Read the model definition and answer for the solid it produces. Units are mm, in the model's axes. Coordinates: 2 decimals unless noted, no trailing zeros. Write each loop counter-clockwise with the first axis right and the second up, starting at its lowest first coordinate (ties: lowest second). Pieces come first, ordered by that corner, then holes.
(1) Find the intervals of material crossed by probe 1 along X at (y, z) = (3.5, 92); probe 2 along Z at (x, y) = (-72, 3.5); probe 3 along X at (y, z) = (3.75, 6.5), in increasing order.
(2) Section C-C on z = 6.5 is taken. Write down the section's boundary in (x, y).
(3) Section D-D on x = 0 is taken. Write down the section's boundary in (y, z).
(4) Section A-A on z = 92 is taken. Write down the section's boundary in (x, y).
(5) Section B-B on x = 72 is taken. Write down the section's boundary in (y, z), then the cut area to 3 significant figures.
(6) Given pin 1 (10 mm diameter, centred on x = 37.5, z = 63.5, fed in from -Y), flat-ended and moving along its own axis, determine where the tip first touches the part or whether it passes through.
from build123d import *

# Parameters (mm, degrees)
SKETCH_1_W               = 170
SKETCH_1_H               = 210
EXTRUDE_1_DEPTH          = 10
CUT_EXTRUDE_1_REACH      = 137.462
SKETCH_2_R               = 9.5
CUT_EXTRUDE_2_REACH      = 137.462
SKETCH_3_R               = 3.5
MIRROR_2_COPY_1_REACH    = 137.462
MIRROR_2_COPY_1_SKETCH_R = 3.5
CHAMFER_1_SIZE           = 2


with BuildPart() as part:
    # 草图1 → 凸台-拉伸1 (new body)
    with BuildSketch(Plane(origin=(0, 0, 0), x_dir=(1, 0, 0), z_dir=(0, 1, 0))):
        Rectangle(SKETCH_1_W, SKETCH_1_H)
    extrude(amount=EXTRUDE_1_DEPTH)

    # 草图2 → 切除-拉伸1 (cut, up to next)
    with BuildSketch(Plane(origin=(0, 10, 0), x_dir=(1, 0, 0), z_dir=(0, 1, 0)), mode=Mode.PRIVATE) as cut_extrude_1_sk1:
        with Locations(Location((0, -6.5, 0), (0, 0, 270))):
            Circle(SKETCH_2_R)
    cut_extrude_1_tool1 = extrude(cut_extrude_1_sk1.sketch, amount=-CUT_EXTRUDE_1_REACH, mode=Mode.PRIVATE) & part.part
    add(cut_extrude_1_tool1.solids().sort_by_distance((0, 10, 6.5))[0], mode=Mode.SUBTRACT)

    # 草图3 → 切除-拉伸2 (cut, up to next)
    with BuildSketch(Plane.XZ, mode=Mode.PRIVATE) as cut_extrude_2_sk1:
        with Locations(Location((72, 92, 0), (0, 0, 270))):
            Circle(SKETCH_3_R)
    cut_extrude_2_tool1 = extrude(cut_extrude_2_sk1.sketch, amount=-CUT_EXTRUDE_2_REACH, mode=Mode.PRIVATE) & part.part
    cut_extrude_2 = cut_extrude_2_tool1.solids().sort_by_distance((72, 0, 92))[0]
    add(cut_extrude_2, mode=Mode.SUBTRACT)

    # 镜向1: 切除-拉伸2 across plane
    add(cut_extrude_2.mirror(Plane(origin=(0, 0, 0), x_dir=(0, 0, 1), z_dir=(1, 0, 0))), mode=Mode.SUBTRACT)

    # 镜向2: 切除-拉伸2 across plane
    add(cut_extrude_2.mirror(Plane.XY), mode=Mode.SUBTRACT)

    # 镜向2 copy 1 sketch → 镜向2 copy 1 (cut, up to next)
    with BuildSketch(Plane(origin=(0, 0, 0), x_dir=(-1, 0, 0), z_dir=(0, -1, 0)), mode=Mode.PRIVATE) as mirror_2_copy_1_sk1:
        with Locations(Location((72, 92, 0), (0, 0, 270))):
            Circle(MIRROR_2_COPY_1_SKETCH_R)
    mirror_2_copy_1_tool1 = extrude(mirror_2_copy_1_sk1.sketch, amount=-MIRROR_2_COPY_1_REACH, mode=Mode.PRIVATE) & part.part
    add(mirror_2_copy_1_tool1.solids().sort_by_distance((-72, 0, -92))[0], mode=Mode.SUBTRACT)

    # 倒角1
    chamfer_1_edges = [part.edges().sort_by_distance(p)[0] for p in [
        (85, 5, 105),
        (-85, 5, 105),
        (-85, 5, -105),
        (85, 5, -105),
    ]]
    chamfer(chamfer_1_edges, length=CHAMFER_1_SIZE)


solid = part.part
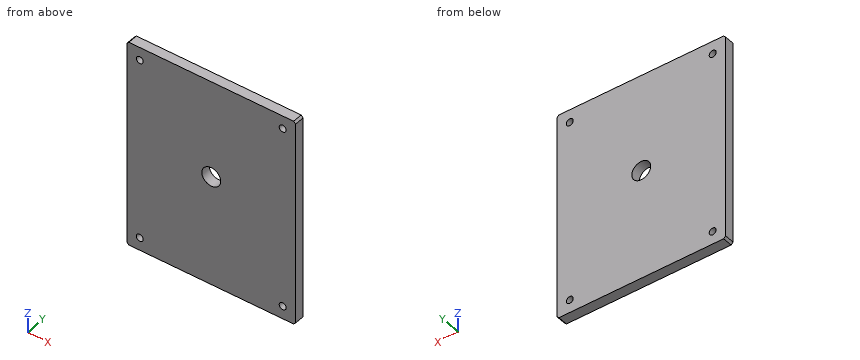
Response:
1. probe 1: x = -85 to -75.5, -68.5 to 68.5, 75.5 to 85
1. probe 2: z = -105 to -95.5, -88.5 to 88.5, 95.5 to 105
1. probe 3: x = -85 to -9.5, 9.5 to 85
2. outline: (-85, 0) - (-9.5, 0) - (-9.5, 10) - (-85, 10) - close; (9.5, 0) - (85, 0) - (85, 10) - (9.5, 10) - close
3. outline: (0, -105) - (10, -105) - (10, -3) - (0, -3) - close; (0, 16) - (10, 16) - (10, 105) - (0, 105) - close
4. outline: (-85, 0) - (-75.5, 0) - (-75.5, 10) - (-85, 10) - close; (-68.5, 0) - (68.5, 0) - (68.5, 10) - (-68.5, 10) - close; (75.5, 0) - (85, 0) - (85, 10) - (75.5, 10) - close
5. outline: (0, -105) - (10, -105) - (10, -95.5) - (0, -95.5) - close; (0, -88.5) - (10, -88.5) - (10, 88.5) - (0, 88.5) - close; (0, 95.5) - (10, 95.5) - (10, 105) - (0, 105) - close
5. area: 1,960 mm2
6. pin 1: stops at y = 0
